Geometry: final body of the model. Coordinates: model frame, mm. Coordinates: 2 decimals unless noted, no trailing zeros. Order: outer loops, then holes, each group sorted by start corner. A loop starts at its lowest first (then second) coordinate and runs counter-clockwise, first axis right, second up. Notation, with made-up numbers: M 12.5,-8 L 41.5,-8 A15 cw 41.5,-3 Z; hole C -39.5,7 d9. An arc over 180 degrees is marked long. One line per question, with ' | ' between items.
from build123d import *

# Parameters (mm, degrees)
SKETCH_1_R          = 30
EXTRUDE_1_DEPTH     = 2
SKETCH_2_R          = 1.6
CUT_EXTRUDE_1_DEPTH = 10
SKETCH_3_R          = 2.55
CUT_EXTRUDE_2_DEPTH = 10
SKETCH_4_R          = 17.5
CUT_EXTRUDE_3_DEPTH = 10
FILLET_1_R          = 3


with BuildPart() as part:
    # 草图1 → 凸台-拉伸1 (new body)
    with BuildSketch(Plane.XY):
        Circle(SKETCH_1_R)
        with BuildLine():
            Line((4, 16.733200531), (4, 12))
            ThreePointArc((4, 12), (4.527864045, 9.763932023), (6, 8))
            ThreePointArc((6, 8), (7.071067812, 7.071067812), (8, 6))
            ThreePointArc((8, 6), (9.763932023, 4.527864045), (12, 4))
            Line((12, 4), (16.733200531, 4))
            ThreePointArc((16.733200531, 4), (21.025175907, 6.43505412), (21.136674355, 11.368421053))
            ThreePointArc((21.136674355, 11.368421053), (16.970562748, 16.970562748), (11.368421053, 21.136674355))
            ThreePointArc((11.368421053, 21.136674355), (6.43505412, 21.025175907), (4, 16.733200531))
        make_face(mode=Mode.SUBTRACT)
        with BuildLine():
            Line((-4, 16.733200531), (-4, 12))
            ThreePointArc((-4, 12), (-4.527864045, 9.763932023), (-6, 8))
            ThreePointArc((-6, 8), (-7.071067812, 7.071067812), (-8, 6))
            ThreePointArc((-8, 6), (-9.763932023, 4.527864045), (-12, 4))
            Line((-12, 4), (-16.733200531, 4))
            ThreePointArc((-16.733200531, 4), (-21.025175907, 6.43505412), (-21.136674355, 11.368421053))
            ThreePointArc((-21.136674355, 11.368421053), (-16.970562748, 16.970562748), (-11.368421053, 21.136674355))
            ThreePointArc((-11.368421053, 21.136674355), (-6.43505412, 21.025175907), (-4, 16.733200531))
        make_face(mode=Mode.SUBTRACT)
        with BuildLine():
            Line((16.733200531, -4), (12, -4))
            ThreePointArc((12, -4), (9.763932023, -4.527864045), (8, -6))
            ThreePointArc((8, -6), (7.071067812, -7.071067812), (6, -8))
            ThreePointArc((6, -8), (4.527864045, -9.763932023), (4, -12))
            Line((4, -12), (4, -16.733200531))
            ThreePointArc((4, -16.733200531), (6.43505412, -21.025175907), (11.368421053, -21.136674355))
            ThreePointArc((11.368421053, -21.136674355), (16.970562748, -16.970562748), (21.136674355, -11.368421053))
            ThreePointArc((21.136674355, -11.368421053), (21.025175907, -6.43505412), (16.733200531, -4))
        make_face(mode=Mode.SUBTRACT)
        with BuildLine():
            Line((-4, -16.733200531), (-4, -12))
            ThreePointArc((-4, -12), (-4.527864045, -9.763932023), (-6, -8))
            ThreePointArc((-6, -8), (-7.071067812, -7.071067812), (-8, -6))
            ThreePointArc((-8, -6), (-9.763932023, -4.527864045), (-12, -4))
            Line((-12, -4), (-16.733200531, -4))
            ThreePointArc((-16.733200531, -4), (-21.025175907, -6.43505412), (-21.136674355, -11.368421053))
            ThreePointArc((-21.136674355, -11.368421053), (-16.970562748, -16.970562748), (-11.368421053, -21.136674355))
            ThreePointArc((-11.368421053, -21.136674355), (-6.43505412, -21.025175907), (-4, -16.733200531))
        make_face(mode=Mode.SUBTRACT)
    extrude(amount=EXTRUDE_1_DEPTH)

    # 草图2 → 切除-拉伸1 (cut)
    with BuildSketch(Plane.XY.offset(2)):
        with Locations((-21, 0)):
            Circle(SKETCH_2_R)
        with Locations((0, 21)):
            Circle(SKETCH_2_R)
        with Locations((21, 0)):
            Circle(SKETCH_2_R)
        with Locations((0, -21)):
            Circle(SKETCH_2_R)
    extrude(amount=-CUT_EXTRUDE_1_DEPTH, mode=Mode.SUBTRACT)

    # 草图3 → 切除-拉伸2 (cut)
    with BuildSketch(Plane.XY.offset(2)):
        with Locations((0, 6)):
            Circle(SKETCH_3_R)
        with Locations((-6, 0)):
            Circle(SKETCH_3_R)
        with Locations((6, 0)):
            Circle(SKETCH_3_R)
        with Locations((0, -6)):
            Circle(SKETCH_3_R)
    extrude(amount=-CUT_EXTRUDE_2_DEPTH, mode=Mode.SUBTRACT)

    # 草图4 → 切除-拉伸3 (cut)
    with BuildSketch(Plane.XY.offset(2)):
        Circle(SKETCH_4_R)
    extrude(amount=-CUT_EXTRUDE_3_DEPTH, mode=Mode.SUBTRACT)

    # 圆角1
    fillet_1_edges = [part.edges().sort_by_distance(p)[0] for p in [
        (-4.009091698, -17.034587866, 1),
        (4.009091698, 17.034587866, 1),
        (17.034587866, 4.009091698, 1),
        (17.034587866, -4.009091698, 1),
        (4.009091698, -17.034587866, 1),
        (-17.034587866, -4.009091698, 1),
        (-17.034587866, 4.009091698, 1),
        (-4.009091698, 17.034587866, 1),
    ]]
    fillet(fillet_1_edges, radius=FILLET_1_R)


solid = part.part
1. Draft query along X for faces 1 (the face through (-29.97, 1.32, 0.99)), 2 (the face through (0, -18, 0)), 3 (the face through (-22.18, 1.08, 1.01)). Return one class per face: pulls with the +X half, pulls with the -X half, needs draft (parallel to the pull), parting line crosses it, or undercut.
Response values:
face 1: parting line crosses it | face 2: needs draft | face 3: undercut
2. Section C-C, the plane x = -13. Output: boundary loops of the cut face in (y, z).
Response values:
outline: M -27.04,0 L -20.17,0 L -20.17,2 L -27.04,2 Z; M 20.17,0 L 27.04,0 L 27.04,2 L 20.17,2 Z
3. Material intervals for line 1 (Y direction, x = 0, z = 1.2); line 2 (X direction, y = -19, z = 1.8); line 3 (Y direction, x = -20.5, z = 0.4), sorted ascending. Write a range as [from, to].
Response values:
line 1: y = [-30, -22.6], [-19.4, -17.5], [17.5, 19.4], [22.6, 30] | line 2: x = [-23.22, -14.66], [-4.54, 4.54], [14.66, 23.22] | line 3: y = [-21.9, -12.48], [-5.71, -1.52], [1.52, 5.71], [12.48, 21.9]
4. Pin query (flat end, axial travel): P1, Ø12, axis at x = -8.5, y = 9.5, coming from the -Z side; P2, Ø1, axis at x = -4.5, z = 0.5, coming from the +Y side. Return the tip coordinate at first contact, or that it passes through.
Response values:
P1: passes through | P2: stops at y = 29.73
5. Section A-A, the plane y = 0. Output: boundary loops of the cut face in (x, z).
Response values:
outline: M -30,0 L -22.6,0 L -22.6,2 L -30,2 Z; M -19.4,0 L -17.5,0 L -17.5,2 L -19.4,2 Z; M 17.5,0 L 19.4,0 L 19.4,2 L 17.5,2 Z; M 22.6,0 L 30,0 L 30,2 L 22.6,2 Z
